```python
from build123d import *

# Parameters (mm, degrees)
SKETCH1_R           = 10
BOSS_EXTRUDE1_DEPTH = 4.5
CUT_EXTRUDE1_START  = -2
SKETCH2_R           = 10
SKETCH2_R_2         = 4.5
CUT_EXTRUDE1_DEPTH  = 2
SKETCH3_R           = 0.75
CUT_EXTRUDE2_DEPTH  = 15.361406616
SKETCH4_R           = 2.95
CUT_EXTRUDE3_DEPTH  = 3.85
SKETCH5_R           = 1.5
CUT_EXTRUDE4_DEPTH  = 15.656824349
M3_TAPPED_HOLE2_D   = 2.5


with BuildPart() as part:
    # Sketch1 → Boss-Extrude1 (new body)
    with BuildSketch(Plane.XY):
        Circle(SKETCH1_R)
    extrude(amount=BOSS_EXTRUDE1_DEPTH)

    # Sketch2 → Cut-Extrude1 (cut)
    with BuildSketch(Plane.XY.offset(4.5).offset(CUT_EXTRUDE1_START)):
        Circle(SKETCH2_R)
        Circle(SKETCH2_R_2, mode=Mode.SUBTRACT)
    extrude(amount=CUT_EXTRUDE1_DEPTH, mode=Mode.SUBTRACT)

    # Sketch3 → Cut-Extrude2 (cut, through all)
    with BuildSketch(Plane.XY.offset(2.5)):
        with Locations((0, 7)):
            Circle(SKETCH3_R)
        with Locations((7, 0)):
            Circle(SKETCH3_R)
        with Locations((0, -7)):
            Circle(SKETCH3_R)
        with Locations((-7, 0)):
            Circle(SKETCH3_R)
    extrude(amount=-CUT_EXTRUDE2_DEPTH, mode=Mode.SUBTRACT)

    # Sketch4 → Cut-Extrude3 (cut)
    with BuildSketch(Plane.XY.offset(4.5)):
        Circle(SKETCH4_R)
    extrude(amount=-CUT_EXTRUDE3_DEPTH, mode=Mode.SUBTRACT)

    # Sketch5 → Cut-Extrude4 (cut, through all)
    with BuildSketch(Plane.XY.offset(0.65)):
        Circle(SKETCH5_R)
    extrude(amount=-CUT_EXTRUDE4_DEPTH, mode=Mode.SUBTRACT)

    # M3 Tapped Hole2 (through all)
    with Locations(Plane.XY.offset(2.5)):
        with Locations((-7, 0), (0, 7), (7, 0), (0, -7)):
            Hole(M3_TAPPED_HOLE2_D / 2)


solid = part.part
```
Model file for the job. Use its own axes, mm. A direction names the side the tool comes from. Coordinates: 2 decimals unless noted, no trailing zeros. Order: outer loops, then holes, each group sorted by start corner. A loop starts at its lowest first (then second) coordinate and runs counter-clockwise, first axis right, second up. Notation, with made-up numbers: (2.25, -22) -> (16.25, -22) arc R16 ccw to (16.25, -16) -> close; hole circle Ø3 at (35.25, -31). An arc over 180 degrees is marked (long way). Return JSON: item names as keys, results as strings.
Item 1: Slice it at D-D (z = 2.25). Write the cut outline in (x, y), then the cut area to 3 significant figures.
Model answer:
{"outline": "circle Ø20 at (0, 0); hole circle Ø2.5 at (-7, 0); hole circle Ø5.9 at (0, 0); hole circle Ø2.5 at (0, -7); hole circle Ø2.5 at (0, 7); hole circle Ø2.5 at (7, 0)", "area": "267 mm²"}
Item 2: Wall check: line 1 along Y through (x, z) = (0, 1.4); line 2 along Y through (x, z) = (0, 2.85); line 3 along Z through (x, y) = (-5.25, -3.5). Give the ranges that are in metal, low to high. Write a range as from..to.
Model answer:
{"line 1": "y = -10..-8.25, -5.75..-2.95, 2.95..5.75, 8.25..10", "line 2": "y = -4.5..-2.95, 2.95..4.5", "line 3": "z = 0..2.5"}
Item 3: Slice it at A-A (y = -6). Write the cut outline in (x, z).
Model answer:
{"outline": "(-8, 0) -> (-0.75, 0) -> (-0.75, 2.5) -> (-8, 2.5) -> close; (0.75, 0) -> (8, 0) -> (8, 2.5) -> (0.75, 2.5) -> close"}
Item 4: Slice it at B-B (y = 0). Write the cut outline in (x, z), then the cut area to 3 significant figures.
Model answer:
{"outline": "(-10, 0) -> (-8.25, 0) -> (-8.25, 2.5) -> (-10, 2.5) -> close; (-5.75, 0) -> (-1.5, 0) -> (-1.5, 0.65) -> (-2.95, 0.65) -> (-2.95, 4.5) -> (-4.5, 4.5) -> (-4.5, 2.5) -> (-5.75, 2.5) -> close; (1.5, 0) -> (5.75, 0) -> (5.75, 2.5) -> (4.5, 2.5) -> (4.5, 4.5) -> (2.95, 4.5) -> (2.95, 0.65) -> (1.5, 0.65) -> close; (8.25, 0) -> (10, 0) -> (10, 2.5) -> (8.25, 2.5) -> close", "area": "30.8 mm²"}
Item 5: 3-axis set-ups, long thin cutter, end or side, ignore diameter. For faces 1 (the face through (-2.947, 0.13, 2.602)), 2 (the face through (-5.75, 0.05, 1.23)): which of +Z, -Z, +X, -X, +Y, -Y reach the whole face in a straight line?
Model answer:
{"face 1": "+Z", "face 2": "+Z, -Z"}
Item 6: Pin check, flat tips, straight feed: P1, Ø1.8, axis at x = -0.5, y = -1, coming from the +Z side; P2, Ø3, axis at x = 0, y = -7, coming from the +Z side; P3, Ø1.5, axis at y = 5, z = 2.5, coming from the -X side. Stop position of each tip, or through.
Model answer:
{"P1": "stops at z = 0.65", "P2": "stops at z = 2.5", "P3": "stops at x = -9.05"}
